from build123d import *

# Parameters (mm, degrees)
SKETCH_1_R             = 4
EXTRUDE_1_DEPTH        = 18
SKETCH_2_R             = 3
EXTRUDE_2_DEPTH        = 50
FILLET_1_R             = 1
CHAMFER_1_SIZE         = 0.5
HOLE_WIZARD_M4_1_D     = 3.3
HOLE_WIZARD_M4_1_DEPTH = 13.5
HOLE_WIZARD_M4_1_TIP   = 0.991420021
SKETCH_5_W             = 2.600851977
SKETCH_5_H             = 9.759387418
SKETCH_5_W_2           = 4.309983276
SKETCH_5_H_2           = 9.585997286
CUT_EXTRUDE_1_DEPTH    = 7


with BuildPart() as part:
    # 草图1 → 凸台-拉伸1 (new body)
    with BuildSketch(Plane.XY):
        Circle(SKETCH_1_R)
    extrude(amount=EXTRUDE_1_DEPTH)

    # 草图2 → 凸台-拉伸2 (add)
    with BuildSketch(Plane.XY.offset(18)):
        Circle(SKETCH_2_R)
    extrude(amount=EXTRUDE_2_DEPTH)

    # 圆角1
    fillet_1_edges = [part.edges().sort_by_distance(p)[0] for p in [
        (-3, 0, 68),
    ]]
    fillet(fillet_1_edges, radius=FILLET_1_R)

    # 倒角1
    chamfer_1_edges = [part.edges().sort_by_distance(p)[0] for p in [
        (-4, 0, 0),
    ]]
    chamfer(chamfer_1_edges, length=CHAMFER_1_SIZE)

    # M4 螺纹孔1
    with Locations(Plane(origin=(0, 0, 0), x_dir=(-1, 0, 0), z_dir=(0, 0, -1))):
        with Locations((0, 0)):
            Hole(HOLE_WIZARD_M4_1_D / 2, depth=HOLE_WIZARD_M4_1_DEPTH)
            with Locations((0, 0, -(HOLE_WIZARD_M4_1_DEPTH + HOLE_WIZARD_M4_1_TIP / 2))):  # 118° drill point
                Cone(0, HOLE_WIZARD_M4_1_D / 2, HOLE_WIZARD_M4_1_TIP, mode=Mode.SUBTRACT)

    # 草图5 → 切除-拉伸1 (cut)
    with BuildSketch(Plane(origin=(0, 0, 3), x_dir=(-1, 0, 0), z_dir=(0, 0, -1))):
        with Locations((-4.800425989, -0.334395254)):
            Rectangle(SKETCH_5_W, SKETCH_5_H)
        with Locations((5.654991638, -0.247700188)):
            Rectangle(SKETCH_5_W_2, SKETCH_5_H_2)
    extrude(amount=-CUT_EXTRUDE_1_DEPTH, mode=Mode.SUBTRACT)


solid = part.part
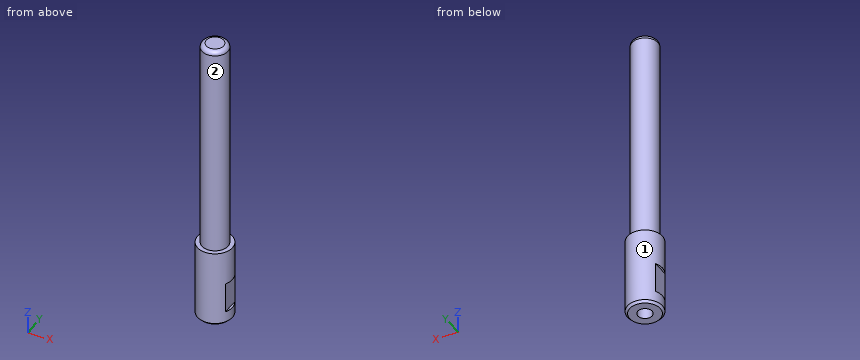
The model under review builds one solid part; all positions refer to its coordinate system, in mm. Face numbers are marked on the shaded views. A direction names the side the tool comes from. Round coordinates to 2 decimals unless told otherwise and drop trailing zeros. Order: outer loops, then holes, each group sorted by start corner. A loop starts at its lowest first (then second) coordinate and runs counter-clockwise, first axis right, second up. Notation, with made-up numbers: (-13, 14.25) -> (3, 14.25) arc R12 cw to (3, 29.25) -> close; hole circle Ø1 at (32.25, 32). An arc over 180 degrees is marked (long way). Use CSV: the item, a comma, the result in double quotes. Start each with the question number.
(1) Insertion check: pin 1 (0.5 mm diameter, centred on x = 4, y = -0.5, fed in from +Z); pin 2 (4.5 mm diameter, centred on y = -0.5, z = 6, fed in from -X); pin 3 (4 mm diameter, centred on x = 2, y = 1.5, fed in from +Z); pin 4 (3 mm diameter, centred on y = 1, z = 5.5, fed in from +X). Each pin has a flat end and moves straight along its axis. Give the tip position at first contact, or say it passes through.
(2) Consider section A-A on z = 37. Write out the cut boundary in (x, y).
(3) Wall thickness on probe 1 along Y at (x, z) = (0, 6.25); probe 2 along X at (y, z) = (0, 3.5); probe 3 along Y at (x, z) = (-0.25, 48.5): over which ranges is each line inside the solid? List them lowest first. Write a range as from..to.
(4) Tool access review of the marked faces 1 and 2: name each direction out of +Z, -Z, +X, -X, +Y, -Y from which nothing blocks a thin tool from reaching the whole face with its end or side.
Responses:
1,pin 1,"z = 18"
1,pin 2,"x = -3.5"
1,pin 3,"z = 68"
1,pin 4,"x = 3.5"
2,outline,"circle Ø6 at (0, 0)"
3,probe 1,"-4..-1.65, 1.65..4"
3,probe 2,"-3.5..-1.65, 1.65..3.5"
3,probe 3,"-2.99..2.99"
4,face 1,"+Z, -Z"
4,face 2,"+Z"
